Design review of the part built by this model. Coordinates are the model's own, in mm. A direction names the side the tool comes from. Give positions to 0.01 mm unless a question says otherwise; leave off trailing zeros. Order: outer loops, then holes, each group sorted by start corner. A loop starts at its lowest first (then second) coordinate and runs counter-clockwise, first axis right, second up.
```python
from build123d import *

# Parameters (mm, degrees)
SKETCH1_W                = 280
SKETCH1_H                = 280
SKETCH1_R                = 75
EXTRUDE1_DEPTH           = 8
SKETCH_2_2_R             = 8.5
SKETCH_2_2_R_2           = 9.5
EXTRUDE2_DEPTH           = 8
EXTRUDE4_START           = -8
SKETCH_2_2_2_R           = 8.5
EXTRUDE4_DEPTH           = 8
EXTRUDE4_DRAFT           = 45
SKETCH_2_2_2_R_2         = 9.5
EXTRUDE4_PROFILE_2_DEPTH = 8
EXTRUDE4_PROFILE_2_DRAFT = 45
EXTRUDE4_PROFILE_3_DEPTH = 8
EXTRUDE4_PROFILE_3_DRAFT = 45
EXTRUDE4_PROFILE_4_DEPTH = 8
EXTRUDE4_PROFILE_4_DRAFT = 45
SKETCH3_W                = 280
SKETCH3_H                = 15
EXTRUDE5_DEPTH           = 16


with BuildPart() as part:
    # Sketch1 → Extrude1 (new, symmetric)
    with BuildSketch(Plane.XY):
        with Locations((0, 24.5)):
            Rectangle(SKETCH1_W, SKETCH1_H)
        Circle(SKETCH1_R, mode=Mode.SUBTRACT)
        with BuildLine():
            Line((-129, 122.5), (-129, 92.5))
            ThreePointArc((-129, 92.5), (-120, 83.5), (-111, 92.5))
            Line((-111, 92.5), (-111, 122.5))
            ThreePointArc((-111, 122.5), (-120, 131.5), (-129, 122.5))
        make_face(mode=Mode.SUBTRACT)
        with BuildLine():
            Line((111, 122.5), (111, 92.5))
            ThreePointArc((111, 92.5), (120, 83.5), (129, 92.5))
            Line((129, 92.5), (129, 122.5))
            ThreePointArc((129, 122.5), (120, 131.5), (111, 122.5))
        make_face(mode=Mode.SUBTRACT)
        with BuildLine():
            Line((-129, -45), (-129, -75))
            ThreePointArc((-129, -75), (-120, -84), (-111, -75))
            Line((-111, -75), (-111, -45))
            ThreePointArc((-111, -45), (-120, -36), (-129, -45))
        make_face(mode=Mode.SUBTRACT)
        with BuildLine():
            Line((111, -45), (111, -75))
            ThreePointArc((111, -75), (120, -84), (129, -75))
            Line((129, -75), (129, -45))
            ThreePointArc((129, -45), (120, -36), (111, -45))
        make_face(mode=Mode.SUBTRACT)
    extrude(amount=EXTRUDE1_DEPTH, both=True)

    # Sketch 2_2 → Extrude2 (cut)
    with BuildSketch(Plane.XY.offset(8)):
        with Locations((-62.578950135, 62.578950135)):
            Circle(SKETCH_2_2_R)
        with Locations((62.578950135, 62.578950135)):
            Circle(SKETCH_2_2_R_2)
        with Locations((62.578950135, -62.578950135)):
            Circle(SKETCH_2_2_R_2)
        with Locations((-62.578950135, -62.578950135)):
            Circle(SKETCH_2_2_R_2)
    extrude(amount=-EXTRUDE2_DEPTH, mode=Mode.SUBTRACT)


with BuildPart() as extrude4_tool:
    # Sketch 2_2 2 → Extrude4 (with draft: the straight prism first)
    with BuildSketch(Plane.XY.offset(8).offset(EXTRUDE4_START)):
        with Locations((-62.578950135, 62.578950135)):
            Circle(SKETCH_2_2_2_R)
    extrude(amount=-EXTRUDE4_DEPTH)
    # Extrude4: the draft: its side faces are tilted about the plane it starts from
    extrude4_sides = [extrude4_tool.faces().sort_by_distance(p)[0] for p in [
        (-71.078950135, 62.578950135, -4),
    ]]
    draft(extrude4_sides, Plane.XY.offset(8).offset(EXTRUDE4_START), EXTRUDE4_DRAFT)


with BuildPart() as part_1:
    add(part.part)

    # Extrude4: cut by extrude4_tool
    add(extrude4_tool.part, mode=Mode.SUBTRACT)


with BuildPart() as extrude4_profile_2_tool:
    # Sketch 2_2 2 → Extrude4 profile 2 (with draft: the straight prism first)
    with BuildSketch(Plane.XY.offset(8).offset(EXTRUDE4_START)):
        with Locations((62.578950135, 62.578950135)):
            Circle(SKETCH_2_2_2_R_2)
    extrude(amount=-EXTRUDE4_PROFILE_2_DEPTH)
    # Extrude4 profile 2: the draft: its side faces are tilted about the plane it starts from
    extrude4_profile_2_sides = [extrude4_profile_2_tool.faces().sort_by_distance(p)[0] for p in [
        (53.078950135, 62.578950135, -4),
    ]]
    draft(extrude4_profile_2_sides, Plane.XY.offset(8).offset(EXTRUDE4_START), EXTRUDE4_PROFILE_2_DRAFT)


with BuildPart() as part_2:
    add(part_1.part)

    # Extrude4 profile 2: cut by extrude4_profile_2_tool
    add(extrude4_profile_2_tool.part, mode=Mode.SUBTRACT)


with BuildPart() as extrude4_profile_3_tool:
    # Sketch 2_2 2 → Extrude4 profile 3 (with draft: the straight prism first)
    with BuildSketch(Plane.XY.offset(8).offset(EXTRUDE4_START)):
        with Locations((62.578950135, -62.578950135)):
            Circle(SKETCH_2_2_2_R_2)
    extrude(amount=-EXTRUDE4_PROFILE_3_DEPTH)
    # Extrude4 profile 3: the draft: its side faces are tilted about the plane it starts from
    extrude4_profile_3_sides = [extrude4_profile_3_tool.faces().sort_by_distance(p)[0] for p in [
        (53.078950135, -62.578950135, -4),
    ]]
    draft(extrude4_profile_3_sides, Plane.XY.offset(8).offset(EXTRUDE4_START), EXTRUDE4_PROFILE_3_DRAFT)


with BuildPart() as part_3:
    add(part_2.part)

    # Extrude4 profile 3: cut by extrude4_profile_3_tool
    add(extrude4_profile_3_tool.part, mode=Mode.SUBTRACT)


with BuildPart() as extrude4_profile_4_tool:
    # Sketch 2_2 2 → Extrude4 profile 4 (with draft: the straight prism first)
    with BuildSketch(Plane.XY.offset(8).offset(EXTRUDE4_START)):
        with Locations((-62.578950135, -62.578950135)):
            Circle(SKETCH_2_2_2_R_2)
    extrude(amount=-EXTRUDE4_PROFILE_4_DEPTH)
    # Extrude4 profile 4: the draft: its side faces are tilted about the plane it starts from
    extrude4_profile_4_sides = [extrude4_profile_4_tool.faces().sort_by_distance(p)[0] for p in [
        (-72.078950135, -62.578950135, -4),
    ]]
    draft(extrude4_profile_4_sides, Plane.XY.offset(8).offset(EXTRUDE4_START), EXTRUDE4_PROFILE_4_DRAFT)


with BuildPart() as part_4:
    add(part_3.part)

    # Extrude4 profile 4: cut by extrude4_profile_4_tool
    add(extrude4_profile_4_tool.part, mode=Mode.SUBTRACT)

    # Sketch3 → Extrude5 (cut)
    with BuildSketch(Plane.XY.offset(8)):
        with Locations((0, -108)):
            Rectangle(SKETCH3_W, SKETCH3_H)
    extrude(amount=-EXTRUDE5_DEPTH, mode=Mode.SUBTRACT)


solid = part_4.part
```
1. Take a section at B-B (y = 110). State the section outline as (x, z) points.
Recorded:
outline: (-140, -8) - (-129, -8) - (-129, 8) - (-140, 8) - close; (-111, -8) - (111, -8) - (111, 8) - (-111, 8) - close; (129, -8) - (140, -8) - (140, 8) - (129, 8) - close
2. Draft analysis for pull direction Y (two halves, no side actions). For faces 3 (the face through (-2, -100.5, 0)), 4 (the face through (-2, 93, 8)), 5 (the face through (-120.198, 83.502, 0.112)), 6 (the face through (71.355, -66.218, 4.056)), state which applies: pulls with the +Y half, pulls with the -Y half, needs draft (parallel to the pull), parting line crosses it, or undercut.
Recorded:
face 3: pulls with the -Y half
face 4: needs draft
face 5: undercut
face 6: undercut
3. Take a section at D-D (z = -4.75). State the section outline as (x, y) points.
Recorded:
outline: (-140, -100.5) - (140, -100.5) - (140, 164.5) - (-140, 164.5) - close; hole (-129, -75) arc R9 ccw to (-111, -75) - (-111, -45) arc R9 ccw to (-129, -45) - close; hole (-129, 92.5) arc R9 ccw to (-111, 92.5) - (-111, 122.5) arc R9 ccw to (-129, 122.5) - close; hole circle Ø26.5 at (-62.58, 62.58); hole (-55.92, -49.98) arc R14.25 ccw (long way) to (-49.98, -55.92) arc R75 ccw to (49.98, -55.92) arc R14.25 ccw (long way) to (55.92, -49.98) arc R75 ccw to (55.92, 49.98) arc R14.25 ccw (long way) to (49.98, 55.92) arc R75 ccw to start; hole (111, -75) arc R9 ccw to (129, -75) - (129, -45) arc R9 ccw to (111, -45) - close; hole (111, 92.5) arc R9 ccw to (129, 92.5) - (129, 122.5) arc R9 ccw to (111, 122.5) - close
4. Machinability: for faces 1 (the face through (119.802, 83.502, 0.112)), 2 (the face through (67.89, 70.92, -0.39)), which of the approach directions +Z, -Z, +X, -X, +Y, -Y give a long, thin tool a straight path to every point of the face, cutting with its end or side? Answer none if there is none.
Recorded:
face 1: +Z, -Z
face 2: -Z
5. Take a section at A-A (x = 120). State the section outline as (y, z) points.
Recorded:
outline: (-100.5, -8) - (-84, -8) - (-84, 8) - (-100.5, 8) - close; (-36, -8) - (83.5, -8) - (83.5, 8) - (-36, 8) - close; (131.5, -8) - (164.5, -8) - (164.5, 8) - (131.5, 8) - close
6. For line 1 along Y through (x, z) = (121, 5.25); line 2 along Y through (x, z) = (-120, -0.5); line 3 along X through (y, z) = (114, 0.75), list the stretches that pass through material, from the lowest coordinate up.
Recorded:
line 1: y = -100.5 to -83.94, -36.06 to 83.56, 131.44 to 164.5
line 2: y = -100.5 to -84, -36 to 83.5, 131.5 to 164.5
line 3: x = -140 to -129, -111 to 111, 129 to 140
7. Take a section at C-C (x = 0). State the section outline as (y, z) points, then the cut area to 3 significant figures.
Recorded:
outline: (-100.5, -8) - (-75, -8) - (-75, 8) - (-100.5, 8) - close; (75, -8) - (164.5, -8) - (164.5, 8) - (75, 8) - close
area: 1,840 mm2
